Input: part model. Units: mm. Frame: model coordinates. Face numbers are marked on the shaded views. A direction names the side the tool comes from. Round coordinates to 2 decimals unless told otherwise and drop trailing zeros. Order: outer loops, then holes, each group sorted by start corner. A loop starts at its lowest first (then second) coordinate and runs counter-clockwise, first axis right, second up. Notation, with made-up numbers: (64.25, 4.5) -> (123.25, 4.5) arc R8 ccw to (123.25, 17.5) -> close; hole circle Ø4 at (77.5, -21.5). An arc over 180 degrees is marked (long way). Use a Markdown table: item, result.
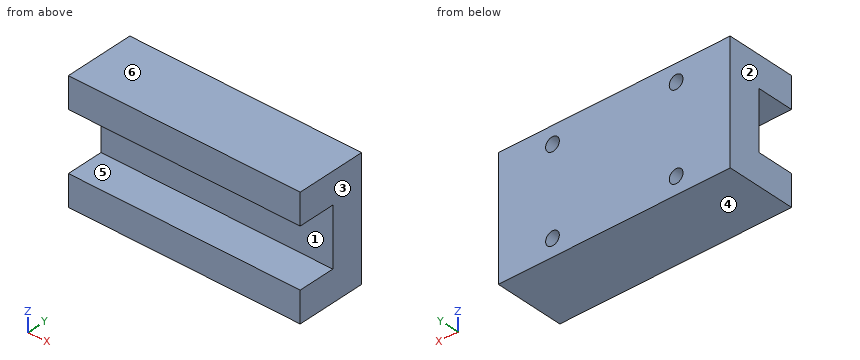
from build123d import *

# Parameters (mm, degrees)
SKETCH_1_W          = 135
SKETCH_1_H          = 70
EXTRUDE_1_DEPTH     = 40.5
SKETCH_2_W          = 135
SKETCH_2_H          = 34
CUT_EXTRUDE_1_DEPTH = 21.5
SKETCH_3_R          = 4
CUT_EXTRUDE_2_DEPTH = 16


with BuildPart() as part:
    # 草图1 → 拉伸1 (new body)
    with BuildSketch(Plane(origin=(0, 0, 0), x_dir=(1, 0, 0), z_dir=(0, 1, 0))):
        with Locations((67.5, 35)):
            Rectangle(SKETCH_1_W, SKETCH_1_H)
    extrude(amount=EXTRUDE_1_DEPTH)

    # 草图2 → 切除-拉伸1 (cut)
    with BuildSketch(Plane.XZ):
        with Locations((67.5, -35)):
            Rectangle(SKETCH_2_W, SKETCH_2_H)
    extrude(amount=-CUT_EXTRUDE_1_DEPTH, mode=Mode.SUBTRACT)

    # 草图3 → 切除-拉伸2 (cut)
    with BuildSketch(Plane(origin=(0, 40.5, 0), x_dir=(-1, 0, 0), z_dir=(0, 1, 0))):
        with Locations(Location((-103.5, -60, 0), (0, 0, 90))):
            Circle(SKETCH_3_R)
        with Locations(Location((-103.5, -10, 0), (0, 0, 90))):
            Circle(SKETCH_3_R)
        with Locations(Location((-31.5, -60, 0), (0, 0, 90))):
            Circle(SKETCH_3_R)
        with Locations(Location((-31.5, -10, 0), (0, 0, 90))):
            Circle(SKETCH_3_R)
    extrude(amount=-CUT_EXTRUDE_2_DEPTH, mode=Mode.SUBTRACT)


solid = part.part
1) Pull-direction query (Z, two-part tool) for the marked faces 3, 4, 5 and 6; classes: +Z half, -Z half, draft (parallel to the pull), parting line (faces both ways), or undercut.
Results found:
| item | result |
|---|---|
| face 3 | draft |
| face 4 | -Z half |
| face 5 | undercut |
| face 6 | +Z half |
2) Cut plane A-A on y = 30. Return loops of the section in (x, z), and give its area (3 significant figures).
Results found:
| item | result |
|---|---|
| outline | (0, -70) -> (135, -70) -> (135, 0) -> (0, 0) -> close; hole circle Ø8 at (31.5, -60); hole circle Ø8 at (31.5, -10); hole circle Ø8 at (103.5, -60); hole circle Ø8 at (103.5, -10) |
| area | 9,250 mm² |
3) Cut plane D-D on y = 11.5. Return loops of the section in (x, z).
Results found:
| item | result |
|---|---|
| outline | (0, -70) -> (135, -70) -> (135, -52) -> (0, -52) -> close; (0, -18) -> (135, -18) -> (135, 0) -> (0, 0) -> close |
4) Pin query (flat end, axial travel): pin 1 Ø5 at (x, z) = (31.5, -60) entering from +Y; pin 2 Ø10 at (x, z) = (57, -31) entering from -Y; pin 3 Ø4 at (x, y) = (75, 18) entering from +Z. Return the tip coordinate at first contact, or that it passes through.
Results found:
| item | result |
|---|---|
| pin 1 | stops at y = 24.5 |
| pin 2 | stops at y = 21.5 |
| pin 3 | stops at z = 0 |
5) Cut plane C-C on x = 113. Return loops of the section in (y, z), and give its area (3 significant figures).
Results found:
| item | result |
|---|---|
| outline | (0, -70) -> (40.5, -70) -> (40.5, 0) -> (0, 0) -> (0, -18) -> (21.5, -18) -> (21.5, -52) -> (0, -52) -> close |
| area | 2,100 mm² |
6) Set-up query: the marked faces 1 and 2. Return all of +Z, -Z, +X, -X, +Y, -Y with unobstructed straight access to the full face (end or side cutting, diameter ignored); none if empty.
Results found:
| item | result |
|---|---|
| face 1 | +X, -X, -Y |
| face 2 | +Z, -Z, -X, +Y, -Y |
7) Cut plane B-B on z = -60. Return loops of the section in (x, y).
Results found:
| item | result |
|---|---|
| outline | (0, 0) -> (135, 0) -> (135, 40.5) -> (107.5, 40.5) -> (107.5, 24.5) -> (99.5, 24.5) -> (99.5, 40.5) -> (35.5, 40.5) -> (35.5, 24.5) -> (27.5, 24.5) -> (27.5, 40.5) -> (0, 40.5) -> close |
8) Line query: L1, parallel to Z at x = 31, y = 33; L2, parallel to X at y = 34, z = -10; L3, parallel to Z at x = 38.5, y = 4.5. Output: solid intervals per line, ascending. Write a range as [from, to].
Results found:
| item | result |
|---|---|
| L1 | z = [-70, -63.97], [-56.03, -13.97], [-6.03, 0] |
| L2 | x = [0, 27.5], [35.5, 99.5], [107.5, 135] |
| L3 | z = [-70, -52], [-18, 0] |
